from build123d import *

# Parameters (mm, degrees)
SKETCH1_R           = 17.5
BOSS_EXTRUDE1_DEPTH = 30
SKETCH2_R           = 21
BOSS_EXTRUDE2_DEPTH = 56.5
SKETCH3_R           = 17.5
BOSS_EXTRUDE3_DEPTH = 273.5
SKETCH4_R           = 15
BOSS_EXTRUDE4_DEPTH = 110
CHAMFER1_SIZE       = 1
CHAMFER3_SIZE       = 1
SKETCH5_W           = 10
SKETCH5_H           = 10
CUT_EXTRUDE1_DEPTH  = 30
CUT_EXTRUDE10_DEPTH = 5.5
CUT_EXTRUDE11_DEPTH = 7


with BuildPart() as part:
    # Sketch1 → Boss-Extrude1 (new body)
    with BuildSketch(Plane(origin=(0, 0, 0), x_dir=(1, 0, 0), z_dir=(0, 1, 0))):
        with Locations(Location((0, 0, 0), (0, 0, 270))):
            Circle(SKETCH1_R)
    extrude(amount=BOSS_EXTRUDE1_DEPTH)

    # Sketch2 → Boss-Extrude2 (add)
    with BuildSketch(Plane(origin=(0, 30, 0), x_dir=(1, 0, 0), z_dir=(0, 1, 0))):
        with Locations(Location((0, 0, 0), (0, 0, 270))):
            Circle(SKETCH2_R)
    extrude(amount=BOSS_EXTRUDE2_DEPTH)

    # Sketch3 → Boss-Extrude3 (add)
    with BuildSketch(Plane(origin=(0, 86.5, 0), x_dir=(1, 0, 0), z_dir=(0, 1, 0))):
        with Locations(Location((0, 0, 0), (0, 0, 270))):
            Circle(SKETCH3_R)
    extrude(amount=BOSS_EXTRUDE3_DEPTH)

    # Sketch4 → Boss-Extrude4 (add)
    with BuildSketch(Plane(origin=(0, 360, 0), x_dir=(1, 0, 0), z_dir=(0, 1, 0))):
        with Locations(Location((0, 0, 0), (0, 0, 270))):
            Circle(SKETCH4_R)
    extrude(amount=BOSS_EXTRUDE4_DEPTH)

    # Chamfer1
    chamfer1_edges = [part.edges().sort_by_distance(p)[0] for p in [
        (0, 0, -17.5),
    ]]
    chamfer(chamfer1_edges, length=CHAMFER1_SIZE)

    # Chamfer3
    chamfer3_edges = [part.edges().sort_by_distance(p)[0] for p in [
        (0, 360, -17.5),
        (0, 470, -15),
        (0, 30, -21),
        (0, 86.5, -21),
    ]]
    chamfer(chamfer3_edges, length=CHAMFER3_SIZE)

    # Sketch5 → Cut-Extrude1 (cut)
    with BuildSketch(Plane.XZ):
        with Locations((0, 17.5)):
            Rectangle(SKETCH5_W, SKETCH5_H)
    extrude(amount=-CUT_EXTRUDE1_DEPTH, mode=Mode.SUBTRACT)

    # Sketch8 → Cut-Extrude10 (cut)
    with BuildSketch(Plane.XY.offset(18)):
        with BuildLine():
            Line((5, 351.5), (5, 322.5))
            ThreePointArc((5, 322.5), (0, 317.5), (-5, 322.5))
            Line((-5, 322.5), (-5, 351.5))
            ThreePointArc((-5, 351.5), (0, 356.5), (5, 351.5))
        make_face()
    extrude(amount=-CUT_EXTRUDE10_DEPTH, mode=Mode.SUBTRACT)

    # Sketch9 → Cut-Extrude11 (cut)
    with BuildSketch(Plane.XY.offset(18)):
        with BuildLine():
            Line((4, 460), (4, 430))
            ThreePointArc((4, 430), (0, 426), (-4, 430))
            Line((-4, 430), (-4, 460))
            ThreePointArc((-4, 460), (0, 464), (4, 460))
        make_face()
    extrude(amount=-CUT_EXTRUDE11_DEPTH, mode=Mode.SUBTRACT)


solid = part.part
Geometry check sheet. Reference: the model listing, model coordinates, mm. A direction names the side the tool comes from. Coordinates: 2 decimals unless noted, no trailing zeros. Order: outer loops, then holes, each group sorted by start corner. A loop starts at its lowest first (then second) coordinate and runs counter-clockwise, first axis right, second up. Notation, with made-up numbers: (17, 58.25) -> (41, 58.25) arc R21 ccw to (41, 66.25) -> close; hole circle Ø4 at (34.25, 35). An arc over 180 degrees is marked (long way). Use a Markdown table: item, result. Add a question column.
1. Set-up check for faces 1 (the face through (-15, 360, 4)), 2 (the face through (0, 445, 11)), 3 (the face through (0, 15, 12.5)): record each of +Z, -Z, +X, -X, +Y, -Y from which the full face is reachable in a straight line by a thin tool's end or side.
2. Material ranges on L1, parallel to X at y = 206, z = 9; L2, parallel to Z at x = 1.5, y = 190.5; L3, parallel to Y at x = 16.5, z = 8.5, recorded low to high.
3. Go/stop test with flat-tipped pins: pin 1 Ø5 at (y, z) = (327.5, 5.5) entering from +X; pin 2 Ø12 at (x, y) = (-7.5, 380) entering from -Z; pin 3 Ø4.5 at (y, z) = (335.5, 15) entering from +X. Record where each tip stops, or that it passes through.
4. Cross-section at B-B (z = 0). Enter the section's corners in (x, y), and give its area (3 significant figures).
5. Cross-section at C-C (y = 437). Enter the section's corners in (x, z).
6. Mould release check, pull along X, two halves, no side actions. Record for faces 4 (the face through (0.66, 413.737, -14.985)), 5 (the face through (0, 470, 0)), 6 (the face through (0, 337, 12.5)): pulls with the +X half, pulls with the -X half, needs draft (parallel to the pull), parting line crosses it, or undercut.
7. Cross-section at D-D (y = 374). Enter the section's corners in (x, z), and give its area (3 significant figures).
Filled sheet:
| question | item | result |
|---|---|---|
| 1 | face 1 | +Y |
| 1 | face 2 | +Z |
| 1 | face 3 | +Z, -Y |
| 2 | L1 | -15.01 to 15.01 |
| 2 | L2 | -17.44 to 17.44 |
| 2 | L3 | 30 to 86.5 |
| 3 | pin 1 | x = 17.24 |
| 3 | pin 2 | z = -14.92 |
| 3 | pin 3 | x = 11.99 |
| 4 | outline | (-21, 31) -> (-20, 30) -> (-17.5, 30) -> (-17.5, 1) -> (-16.5, 0) -> (16.5, 0) -> (17.5, 1) -> (17.5, 30) -> (20, 30) -> (21, 31) -> (21, 85.5) -> (20, 86.5) -> (17.5, 86.5) -> (17.5, 359) -> (16.5, 360) -> (15, 360) -> (15, 469) -> (14, 470) -> (-14, 470) -> (-15, 469) -> (-15, 360) -> (-16.5, 360) -> (-17.5, 359) -> (-17.5, 86.5) -> (-20, 86.5) -> (-21, 85.5) -> close |
| 4 | area | 16,300 mm2 |
| 5 | outline | (-4, 11) -> (-4, 14.46) arc R15 ccw (long way) to (4, 14.46) -> (4, 11) -> close |
| 6 | face 4 | parting line crosses it |
| 6 | face 5 | needs draft |
| 6 | face 6 | undercut |
| 7 | outline | circle Ø30 at (0, 0) |
| 7 | area | 707 mm2 |
